```python
from build123d import *


with BuildPart() as part:
    # Sketch1 → Revolve1 (revolve)
    with BuildSketch(Plane.XY, mode=Mode.PRIVATE) as revolve1_sk:
        with BuildLine():
            Line((37.5, 92.5), (25, 92.5))
            Line((25, 92.5), (25, 25.700367412))
            Line((25, 25.700367412), (41.295159506, -89.5))
            Line((41.295159506, -89.5), (50, -89.5))
            Line((50, -89.5), (50, -92.5))
            Line((50, -92.5), (70, -92.5))
            Line((70, -92.5), (70, -72.5))
            Line((70, -72.5), (54.342520005, -72.5))
            ThreePointArc((54.342520005, -72.5), (51.063908223, -71.275010567), (49.391802356, -68.200281914))
            Line((49.391802356, -68.200281914), (33.044354116, 47.369746278))
            ThreePointArc((33.044354116, 47.369746278), (34.102490489, 50.950750604), (37.5, 52.5))
            Line((37.5, 52.5), (37.5, 92.5))
        make_face()
    revolve(revolve1_sk.sketch.rotate(Axis((0, 92.5, 0), (0, -1, 0)), 180), axis=Axis((0, 92.5, 0), (0, -1, 0)))


solid = part.part
```
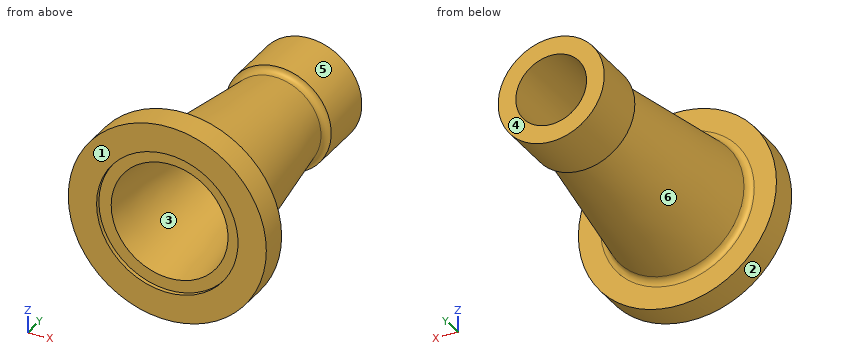
Can you work these out from the model? Positions are in its coordinate system, mm. Face numbers are marked on the shaded views. A direction names the side the tool comes from. Round coordinates to 2 decimals unless told otherwise and drop trailing zeros. Order: outer loops, then holes, each group sorted by start corner. A loop starts at its lowest first (then second) coordinate and runs counter-clockwise, first axis right, second up. Notation, with made-up numbers: (-30, 65.5) -> (18, 65.5) arc R29 cw to (18, 86.5) -> close; hole circle Ø6 at (3.5, 2). An arc over 180 degrees is marked (long way). Return JSON: item names as keys, results as strings. Group by question number.
1. If we section it at A-A, the plane z = 0: Write out the boundary of the cut face in (x, y), then the cut area to 3 significant figures.
2. Will these pins go through, and if not, where does the flat tip stop? pin 1 (6 mm diameter, centred on y = 33, z = -7, fed in from +X); pin 2 (1.5 mm diameter, centred on x = 30.5, y = 65, fed in from -Z); pin 3 (5 mm diameter, centred on x = 32, y = -72.5, fed in from +Z).
3. If we section it at D-D, the plane z = 58: Write out the boundary of the cut face in (x, y), then the cut area to 3 significant figures.
4. We'd pull the mould along Z, two halves only. Please class the marked faces 1, 2 and 3: released by +Z, released by -Z, zero draft, split by the parting line, or undercut.
5. Which directions (+Z, -Z, +X, -X, +Y, -Y) give clear straight access to the entire face, cutting with the end or side of a thin tool? Please do the marked faces 4, 5 and 6.
6. I need wall thicknesses on line 1 (Z direction, x = 0, y = 71.5); line 2 (Z direction, x = 0, y = -90); line 3 (Y direction, x = 57, z = 21). Which ranges of each line are inside material? Lowest first, please. Write a range as [from, to].
7. If we section it at B-B, the plane x = 0: Write out the boundary of the cut face in (y, z).
8. If we section it at C-C, the plane y = 3: Write out the boundary of the cut face in (x, z), then the cut area to 3 significant figures.
Output values:
{
 "1": {"outline": "(-70, -92.5) -> (-50, -92.5) -> (-50, -89.5) -> (-41.3, -89.5) -> (-25, 25.7) -> (-25, 92.5) -> (-37.5, 92.5) -> (-37.5, 52.5) arc R4.5 cw to (-33.04, 47.37) -> (-49.39, -68.2) arc R5 cw to (-54.34, -72.5) -> (-70, -72.5) -> close; (25, 25.7) -> (41.3, -89.5) -> (50, -89.5) -> (50, -92.5) -> (70, -92.5) -> (70, -72.5) -> (54.34, -72.5) arc R5 cw to (49.39, -68.2) -> (33.04, 47.37) arc R4.5 cw to (37.5, 52.5) -> (37.5, 92.5) -> (25, 92.5) -> close", "area": "4,830 mm²"},
 "2": {"pin 1": "x = 35.04", "pin 2": "z = -22.83", "pin 3": "z = 63.48"},
 "3": {"outline": "(-39.19, -92.5) -> (39.19, -92.5) -> (39.19, -72.5) -> (-39.19, -72.5) -> close", "area": "1,570 mm²"},
 "4": {"face 1": "zero draft", "face 2": "split by the parting line", "face 3": "undercut"},
 "5": {"face 4": "+Z, -Z, +X, -X, +Y", "face 5": "+Y", "face 6": "none"},
 "6": {"line 1": "[-37.5, -25], [25, 37.5]", "line 2": "[-70, -50], [50, 70]", "line 3": "[-92.5, -72.5]"},
 "7": {"outline": "(-92.5, -70) -> (-72.5, -70) -> (-72.5, -54.34) arc R5 cw to (-68.2, -49.39) -> (47.37, -33.04) arc R4.5 cw to (52.5, -37.5) -> (92.5, -37.5) -> (92.5, -25) -> (25.7, -25) -> (-89.5, -41.3) -> (-89.5, -50) -> (-92.5, -50) -> close; (-92.5, 50) -> (-89.5, 50) -> (-89.5, 41.3) -> (25.7, 25) -> (92.5, 25) -> (92.5, 37.5) -> (52.5, 37.5) arc R4.5 cw to (47.37, 33.04) -> (-68.2, 49.39) arc R5 cw to (-72.5, 54.34) -> (-72.5, 70) -> (-92.5, 70) -> close"},
 "8": {"outline": "circle Ø78.64 at (0, 0); hole circle Ø56.42 at (0, 0)", "area": "2,360 mm²"}
}
